Design review of the part shown in the three views and the two pictorial views. Dimensions are in mm from the part's minimum x, y and z. A direction names the side the tool comes from. Give positions to 0.01 mm unless a question says otherwise; leave off trailing zeros. Order: outer loops, then holes, each group sorted by start corner. A loop starts at its lowest first (then second) coordinate and runs counter-clockwise, first axis right, second up. Notation, with made-up numbers: (-36.75, -17.5) -> (-28.75, -17.5) arc R20 cw to (-28.75, 18.5) -> close; hole circle Ø10 at (33, 70). An arc over 180 degrees is marked (long way). Answer in a Markdown table with one row per item. Add a question column.
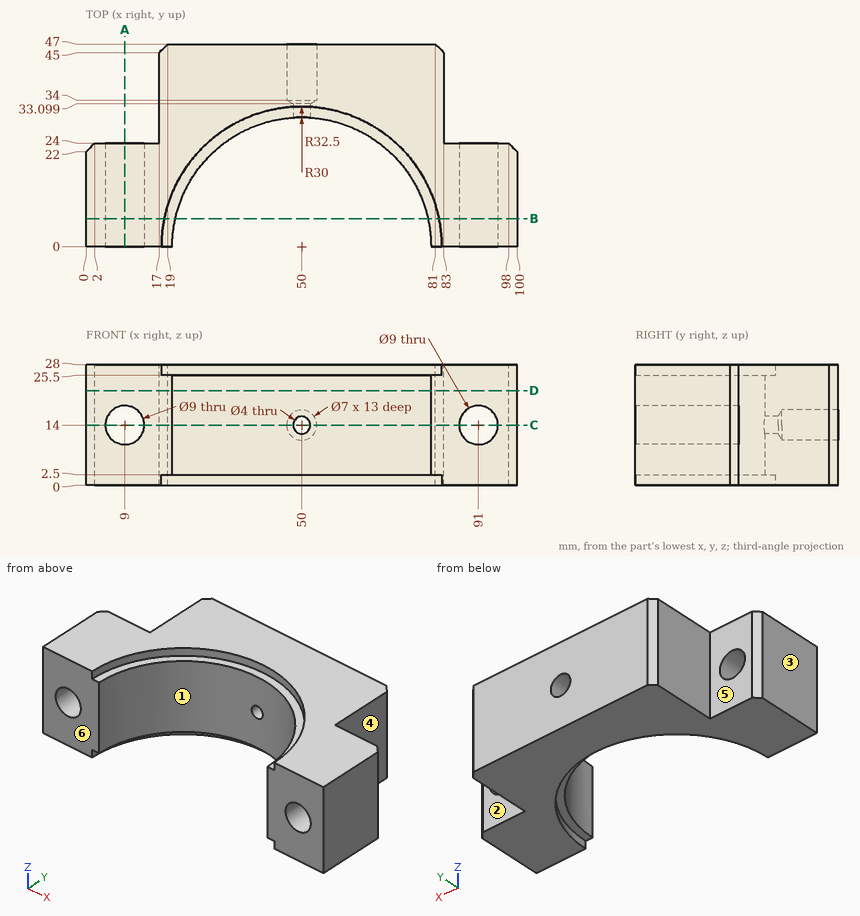
1) Add section A-A, the plane x = 9. Write out the cut boundary in (y, z).
2) Mouldability with a two-part tool opening along X and no side actions: class the marked faces 1, 2 and 3 as +X half, -X half, draft (parallel to the pull), parting line (faces both ways), or undercut.
3) For L1, parallel to X at y = 44, z = 14; L2, parallel to X at y = 11, z = 14.75; L3, parallel to Z at x = 50, y = 39.5, list the stretches that pass through material, from the lowest coordinate up.
4) Add section D-D, the plane z = 22. Write out the cut boundary in (x, y), and give its area (3 significant figures).
5) Machinability: for the marked faces 4, 5 and 6, which of the approach directions +Z, -Z, +X, -X, +Y, -Y give a long, thin tool a straight path to every point of the face, cutting with its end or side? Answer none if there is none.
6) Add section B-B, the plane y = 6.5. Write out the cut boundary in (x, z).
7) Add section C-C, the plane z = 14. Give the number of separate pieces and of enclosed holes in the cut face, and give its area (3 significant figures).
8) Clearance check with flat-ended pins moving along their axes: P1, Ø3, axis at x = 42.5, z = 5.5, coming from the -Y side; P2, Ø6.5, axis at y = 33, z = 8.5, coming from the +X side; P3, Ø4.5, axis at x = 94, z = 12, coming from the +Y side. State where each tip first meets the part, or that it passes through.
Verdict:
| question | item | result |
|---|---|---|
| 1 | outline | (0, 0) -> (24, 0) -> (24, 9.5) -> (0, 9.5) -> close; (0, 18.5) -> (24, 18.5) -> (24, 28) -> (0, 28) -> close |
| 2 | face 1 | undercut |
| 2 | face 2 | draft |
| 2 | face 3 | -X half |
| 3 | L1 | x = 17 to 46.5, 53.5 to 83 |
| 3 | L2 | x = 0 to 4.56, 13.44 to 22.09, 77.91 to 86.56, 95.44 to 100 |
| 3 | L3 | z = 0 to 10.5, 17.5 to 28 |
| 4 | outline | (0, 0) -> (20, 0) arc R30 cw to (80, 0) -> (100, 0) -> (100, 22) -> (98, 24) -> (83, 24) -> (83, 45) -> (81, 47) -> (19, 47) -> (17, 45) -> (17, 24) -> (2, 24) -> (0, 22) -> close |
| 4 | area | 2,500 mm2 |
| 5 | face 4 | +Z, -Z, +X, +Y |
| 5 | face 5 | +Z, -Z, -X, +Y |
| 5 | face 6 | +Z, -Z, +X, -X, -Y |
| 6 | outline | (0, 0) -> (18.16, 0) -> (18.16, 2.5) -> (20.71, 2.5) -> (20.71, 25.5) -> (18.16, 25.5) -> (18.16, 28) -> (0, 28) -> close; (79.29, 2.5) -> (81.84, 2.5) -> (81.84, 0) -> (100, 0) -> (100, 28) -> (81.84, 28) -> (81.84, 25.5) -> (79.29, 25.5) -> close; hole circle Ø9 at (9, 14); hole circle Ø9 at (91, 14) |
| 7 | separate pieces | 4 |
| 7 | enclosed holes | 0 |
| 7 | area | 1,960 mm2 |
| 8 | P1 | stops at y = 28.62 |
| 8 | P2 | stops at x = 83 |
| 8 | P3 | stops at y = 24 |
